Geometry: final body of the model. Coordinates: model frame, mm. A direction names the side the tool comes from. Round coordinates to 2 decimals unless told otherwise and drop trailing zeros. Write each loop counter-clockwise with the first axis right and the second up, starting at its lowest first coordinate (ties: lowest second). Pieces come first, ordered by that corner, then holes. Notation, with made-up numbers: (52, 77.25) -> (103, 77.25) arc R31 cw to (103, 116.25) -> close; hole circle Ø2 at (37, -17). An arc over 180 degrees is marked (long way). Use one line per item in the form item = value. Start each with the question number.
1. Reachability of faces 1 (the face through (-40.11, 4.04, 6.38)), 2 (the face through (31.6, 0.86, 2.46)), 3 (the face through (0, 0.2, 5)) from +Z, -Z, +X, -X, +Y, -Y: full face, straight path, thin tool, end or side. Return the list, or none.
2. Cut plane B-B, the plane x = -12.5. Return the cut outline in (y, z).
3. Line query: L1, parallel to X at y = 5, z = 4.5; L2, parallel to Y at x = 14, z = -1.75; L3, parallel to X at y = 5, z = 9.75. Output: solid intervals per line, ascending.
4. Draft query along Y for faces 4 (the face through (-30, 5, -2)), 5 (the face through (-42.5, 5, 5)), 6 (the face through (31.6, 9.14, 2.46)). Return one class per face: pulls with the +Y half, pulls with the -Y half, needs draft (parallel to the pull), parting line crosses it, or undercut.
5. Cut plane A-A, the plane z = 8.5. Return the cut outline in (x, y), plus the area to 3 significant figures.
6. Pin query (flat end, axial travel): pin 1 Ø3 at (x, y) = (-23, 5) entering from +Z; pin 2 Ø1 at (x, y) = (32.5, 3) entering from +Z; pin 3 Ø4 at (y, z) = (6.5, 8) entering from +X; pin 4 Ø5 at (x, y) = (13.5, 4.5) entering from +Z. Return the tip coordinate at first contact, or that it passes through.
7. Cut plane C-C, the plane z = 2.25. Return the cut outline in (x, y), plus the area to 3 significant figures.
```python
from build123d import *

# Parameters (mm, degrees)
SKETCH1_W             = 85
SKETCH1_H             = 10
BOSS_EXTRUDE1_DEPTH   = 10
CUT_EXTRUDE1_DEPTH    = 4.4
CUT_EXTRUDE2_DEPTH    = 45.018291652
SKETCH4_W             = 9.4
SKETCH4_H             = 10
BOSS_EXTRUDE2_DEPTH   = 10
SKETCH5_W             = 10
SKETCH5_H             = 10
CUT_EXTRUDE3_DEPTH    = 5
M6_TAPPED_HOLE1_D     = 5
M6_TAPPED_HOLE1_DEPTH = 17
M6_TAPPED_HOLE1_TIP   = 1.502151548
M4_TAPPED_HOLE1_D     = 3.3
M4_TAPPED_HOLE1_DEPTH = 11.5
M4_TAPPED_HOLE1_TIP   = 0.991420021
FILLET1_R             = 3
CHAMFER2_SIZE         = 1
FILLET2_R             = 1
CHAMFER3_SIZE         = 1
FILLET3_R             = 3


with BuildPart() as part:
    # Sketch1 → Boss-Extrude1 (new body)
    with BuildSketch(Plane(origin=(0, 0, 0), x_dir=(1, 0, 0), z_dir=(0, 1, 0))):
        Rectangle(SKETCH1_W, SKETCH1_H)
    extrude(amount=BOSS_EXTRUDE1_DEPTH)

    # Sketch2 → Cut-Extrude1 (cut)
    with BuildSketch(Plane.XY.offset(5)):
        with BuildLine():
            Line((-27.75, 9), (27.75, 9))
            ThreePointArc((27.75, 9), (31.75, 5), (27.75, 1))
            Line((27.75, 1), (-27.75, 1))
            ThreePointArc((-27.75, 1), (-31.75, 5), (-27.75, 9))
        make_face()
    extrude(amount=-CUT_EXTRUDE1_DEPTH, mode=Mode.SUBTRACT)

    # Sketch3 → Cut-Extrude2 (cut, through all)
    with BuildSketch(Plane.XY.offset(0.6)):
        with BuildLine():
            Line((-27.75, 7.25), (27.75, 7.25))
            ThreePointArc((27.75, 7.25), (30, 5), (27.75, 2.75))
            Line((27.75, 2.75), (-27.75, 2.75))
            ThreePointArc((-27.75, 2.75), (-30, 5), (-27.75, 7.25))
        make_face()
    extrude(amount=-CUT_EXTRUDE2_DEPTH, mode=Mode.SUBTRACT)

    # Sketch4 → Boss-Extrude2 (add)
    with BuildSketch(Plane.XY.offset(5)):
        with Locations((-37.8, 5)):
            Rectangle(SKETCH4_W, SKETCH4_H)
    extrude(amount=BOSS_EXTRUDE2_DEPTH)

    # Sketch5 → Cut-Extrude3 (cut)
    with BuildSketch(Plane.XY.offset(5)):
        with Locations((37.5, 5)):
            Rectangle(SKETCH5_W, SKETCH5_H)
    extrude(amount=-CUT_EXTRUDE3_DEPTH, mode=Mode.SUBTRACT)

    # M6 Tapped Hole1
    with Locations(Plane.XY.offset(15)):
        with Locations((-37.8, 5)):
            Hole(M6_TAPPED_HOLE1_D / 2, depth=M6_TAPPED_HOLE1_DEPTH)
            with Locations((0, 0, -(M6_TAPPED_HOLE1_DEPTH + M6_TAPPED_HOLE1_TIP / 2))):  # 118° drill point
                Cone(0, M6_TAPPED_HOLE1_D / 2, M6_TAPPED_HOLE1_TIP, mode=Mode.SUBTRACT)

    # M4 Tapped Hole1
    with Locations(Plane.XY):
        with Locations((37.5, 5.5)):
            Hole(M4_TAPPED_HOLE1_D / 2, depth=M4_TAPPED_HOLE1_DEPTH)
            with Locations((0, 0, -(M4_TAPPED_HOLE1_DEPTH + M4_TAPPED_HOLE1_TIP / 2))):  # 118° drill point
                Cone(0, M4_TAPPED_HOLE1_D / 2, M4_TAPPED_HOLE1_TIP, mode=Mode.SUBTRACT)

    # Fillet1
    fillet1_edges = [part.edges().sort_by_distance(p)[0] for p in [
        (32.5, 0, 2.5),
        (32.5, 10, 2.5),
    ]]
    fillet(fillet1_edges, radius=FILLET1_R)

    # Chamfer2
    chamfer2_edges = [part.edges().sort_by_distance(p)[0] for p in [
        (-37.8, 10, 15),
        (-33.1, 5, 15),
        (-42.5, 5, 15),
        (-37.8, 0, 15),
    ]]
    chamfer(chamfer2_edges, length=CHAMFER2_SIZE)

    # Fillet2
    fillet2_edges = [part.edges().sort_by_distance(p)[0] for p in [
        (-33.1, 5, 5),
    ]]
    fillet(fillet2_edges, radius=FILLET2_R)

    # Chamfer3
    chamfer3_edges = [part.edges().sort_by_distance(p)[0] for p in [
        (0, 10, -5),
        (-42.5, 10, 4.5),
        (0, 0, -5),
        (-42.5, 0, 4.5),
        (-42.5, 5, -5),
    ]]
    chamfer(chamfer3_edges, length=CHAMFER3_SIZE)

    # Fillet3
    fillet3_edges = [part.edges().sort_by_distance(p)[0] for p in [
        (42.5, 0, -2),
        (42.5, 10, -2),
    ]]
    fillet(fillet3_edges, radius=FILLET3_R)


solid = part.part
```
Outcome:
q1.face_1 = +Z
q1.face_2 = +Z, +X, -Y
q1.face_3 = +Z, +X, +Y, -Y
q2.outline = (0, -4) -> (1, -5) -> (2.75, -5) -> (2.75, 0.6) -> (1, 0.6) -> (1, 5) -> (0, 5) -> close; (7.25, -5) -> (9, -5) -> (10, -4) -> (10, 5) -> (9, 5) -> (9, 0.6) -> (7.25, 0.6) -> close
q3.L1 = -42.5 to -40.3, -35.3 to -31.75, 31.75 to 32.5
q3.L2 = 0 to 2.75, 7.25 to 10
q3.L3 = -42.5 to -40.3, -35.3 to -33.1
q4.face_4 = undercut
q4.face_5 = needs draft
q4.face_6 = pulls with the +Y half
q5.outline = (-42.5, 1) -> (-41.5, 0) -> (-33.1, 0) -> (-33.1, 10) -> (-41.5, 10) -> (-42.5, 9) -> close; hole circle Ø5 at (-37.8, 5)
q5.area = 73.4 mm^2
q6.pin_1 = through
q6.pin_2 = 5
q6.pin_3 = -33.1
q6.pin_4 = 0.6
q7.outline = (-42.5, 1) -> (-41.5, 0) -> (29.5, 0) arc R3 ccw to (32.5, 3) -> (32.5, 7) arc R3 ccw to (29.5, 10) -> (-41.5, 10) -> (-42.5, 9) -> close; hole circle Ø5 at (-37.8, 5); hole (-27.75, 1) -> (27.75, 1) arc R4 ccw to (27.75, 9) -> (-27.75, 9) arc R4 ccw to start
q7.area = 231 mm^2
